Model file for the job. Use its own axes, mm. A direction names the side the tool comes from. Round coordinates to 2 decimals unless told otherwise and drop trailing zeros. Loops run counter-clockwise (first coordinate to the right, second up) from the corner with the lowest first, then second, coordinate; pieces in that order, holes last. Notation, with made-up numbers: (-30.5, -8.75) - (7.5, -8.75) arc R11 ccw to (7.5, 8.25) - close; hole circle Ø6 at (62, 64.25). An arc over 180 degrees is marked (long way). Use one line per item in the form item = value.
from build123d import *

# Parameters (mm, degrees)
SKETCH_1_W                = 150
SKETCH_1_H                = 150
EXTRUDE_1_DEPTH           = 15
HOLE_WIZARD_1_D           = 9
HOLE_WIZARD_1_CBORE_D     = 15
HOLE_WIZARD_1_CBORE_DEPTH = 9


with BuildPart() as part:
    # 草图1 → 凸台-拉伸1 (new body)
    with BuildSketch(Plane(origin=(0, 0, 0), x_dir=(0, 0, -1), z_dir=(1, 0, 0))):
        Rectangle(SKETCH_1_W, SKETCH_1_H)
    extrude(amount=EXTRUDE_1_DEPTH)

    # 打孔尺寸(%根据)内六角圆柱头螺钉的类型1 (through all)
    with Locations(Plane(origin=(15, 0, 0), x_dir=(0, 0, -1), z_dir=(1, 0, 0))):
        with Locations((-40, 50), (40, 50), (-40, -50), (40, -50)):
            CounterBoreHole(HOLE_WIZARD_1_D / 2, HOLE_WIZARD_1_CBORE_D / 2, HOLE_WIZARD_1_CBORE_DEPTH)


solid = part.part
1. Wall check: probe 1 along Y at (x, z) = (2.7, -40); probe 2 along Y at (x, z) = (10.25, -40); probe 3 along Z at (x, y) = (7.5, 50.5). Give the ranges that are in metal, low to high.
Geometry check:
probe_1 = -75 to -54.5, -45.5 to 45.5, 54.5 to 75
probe_2 = -75 to -57.5, -42.5 to 42.5, 57.5 to 75
probe_3 = -75 to -47.48, -32.52 to 32.52, 47.48 to 75
2. Cut at A-A, the plane x = 10.25. Give the cut face in (y, z).
Geometry check:
outline = (-75, -75) - (75, -75) - (75, 75) - (-75, 75) - close; hole circle Ø15 at (-50, -40); hole circle Ø15 at (-50, 40); hole circle Ø15 at (50, -40); hole circle Ø15 at (50, 40)
3. Flat gauge pins, fed straight in: pin 1 (7.5 mm diameter, centred on y = -48, z = -40, fed in from +X); pin 2 (19.5 mm diameter, centred on y = 50, z = -40, fed in from -X). Where does each tip first touch, or does it go through?
Geometry check:
pin_1 = 6
pin_2 = 0
4. Pull direction Z, two halves, no side cores. Call faces 1 (the cylindrical face through (2.96, -53.99, -37.92)), 2 (the flat face through (7, -1, -75)), 3 (the flat face through (7, -1, 75)), 4 (the flat face through (7, 75, 1)): +Z half, -Z half, draft (parallel to the pull), parting line (faces both ways), or undercut.
Geometry check:
face_1 = undercut
face_2 = -Z half
face_3 = +Z half
face_4 = draft
5. Cut at C-C, the plane y = 50. Give the cut face in (x, z), plus the area to 3 significant figures.
Geometry check:
outline = (0, -75) - (15, -75) - (15, -47.5) - (6, -47.5) - (6, -44.5) - (0, -44.5) - close; (0, -35.5) - (6, -35.5) - (6, -32.5) - (15, -32.5) - (15, 32.5) - (6, 32.5) - (6, 35.5) - (0, 35.5) - close; (0, 44.5) - (6, 44.5) - (6, 47.5) - (15, 47.5) - (15, 75) - (0, 75) - close
area = 1,870 mm^2
6. Tool access for faces 5 (the flat face through (6, 45, 40)), 6 (the cylindrical face through (2.96, 46.01, 42.08)): list every direction of +Z, -Z, +X, -X, +Y, -Y with a clear straight run to the whole face (end or side of a thin tool).
Geometry check:
face_5 = +X
face_6 = +X, -X
7. Cut at B-B, the plane z = 40. Give the cut face in (x, y).
Geometry check:
outline = (0, -75) - (15, -75) - (15, -57.5) - (6, -57.5) - (6, -54.5) - (0, -54.5) - close; (0, -45.5) - (6, -45.5) - (6, -42.5) - (15, -42.5) - (15, 42.5) - (6, 42.5) - (6, 45.5) - (0, 45.5) - close; (0, 54.5) - (6, 54.5) - (6, 57.5) - (15, 57.5) - (15, 75) - (0, 75) - close
